The figure shows three views and two pictorial views of one solid part (mm, origin at its lowest corner). Answer the questions. Round coordinates to 2 decimals unless told otherwise and drop trailing zeros. Order: outer loops, then holes, each group sorted by start corner. A loop starts at its lowest first (then second) coordinate and runs counter-clockwise, first axis right, second up. Notation, with made-up numbers: (26.25, 83.5) - (47.25, 83.5) arc R19 cw to (47.25, 88.5) - close; hole circle Ø1 at (42, 57). An arc over 180 degrees is marked (long way). Answer as a JSON object with one key per item and string values. Group by question number.
Q1. A cutting plane is placed at C-C on y = 7.5. Determine the outline of the cut face in (x, z).
Q2. Given pin 1 Ø4 at (x, y) = (15.5, 17.5) entering from -Z, flat-ended and moving along its own axis, determine where the tip first touches the part or whether it passes through.
Q3. A cutting plane is placed at D-D on x = 20. Determine the outline of the cut face in (y, z).
Q4. A cutting plane is placed at B-B on z = 8.5. Determine the outline of the cut face in (x, y).
Q5. Consider line 1 (X direction, y = 12, z = 8.5); line 2 (X direction, y = 9.25, z = 5); line 3 (Z direction, x = 32, y = 12.25). Determine where each line is inside the solid, lowest interval first.
Q6. The mould has two halves that part along X. Classify the marked faces 1, 2, 3 and 4: pulls with the +X half, pulls with the -X half, needs draft (parallel to the pull), parting line crosses it, or undercut.
Q7. A cutting plane is placed at A-A on x = 33. Determine the outline of the cut face in (y, z), and give its area (3 significant figures).
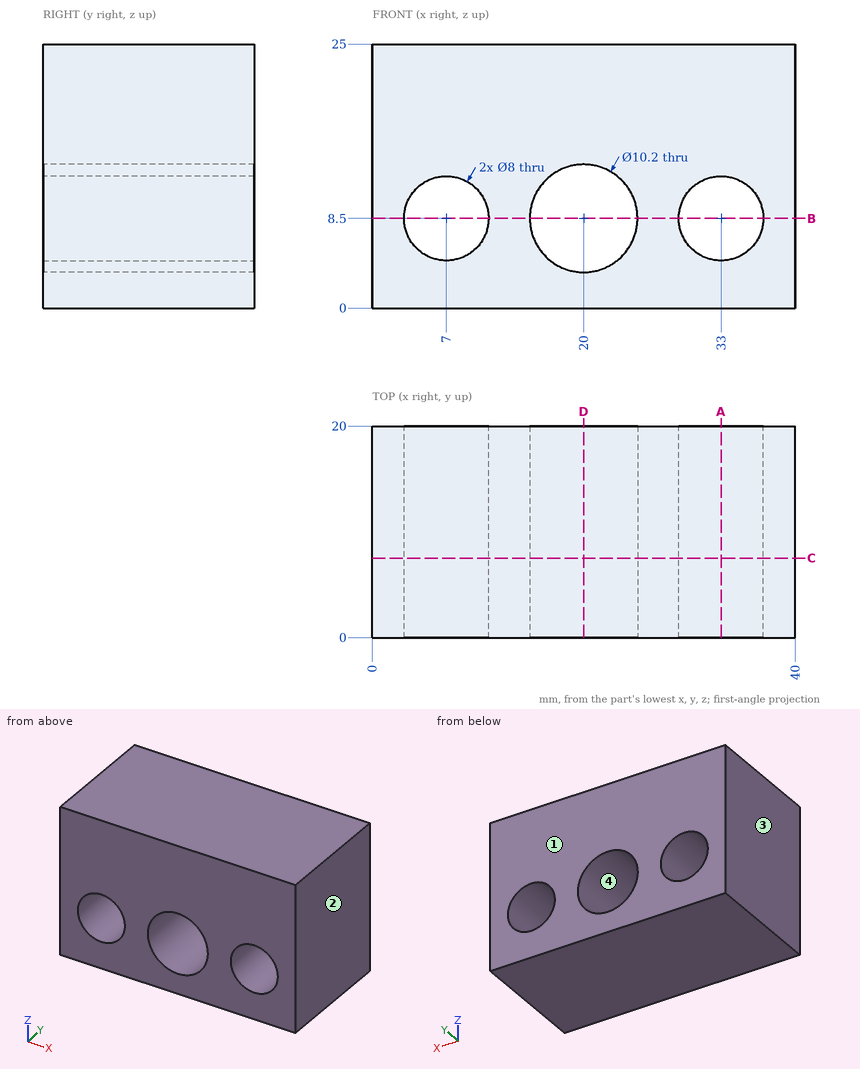
Result set:
{
 "1": {"outline": "(0, 0) - (40, 0) - (40, 25) - (0, 25) - close; hole circle Ø8 at (7, 8.5); hole circle Ø10.2 at (20, 8.5); hole circle Ø8 at (33, 8.5)"},
 "2": {"pin 1": "stops at z = 0"},
 "3": {"outline": "(0, 0) - (20, 0) - (20, 3.4) - (0, 3.4) - close; (0, 13.6) - (20, 13.6) - (20, 25) - (0, 25) - close"},
 "4": {"outline": "(0, 0) - (3, 0) - (3, 20) - (0, 20) - close; (11, 0) - (14.9, 0) - (14.9, 20) - (11, 20) - close; (25.1, 0) - (29, 0) - (29, 20) - (25.1, 20) - close; (37, 0) - (40, 0) - (40, 20) - (37, 20) - close"},
 "5": {"line 1": "x = 0 to 3, 11 to 14.9, 25.1 to 29, 37 to 40", "line 2": "x = 0 to 5.06, 8.94 to 16.29, 23.71 to 31.06, 34.94 to 40", "line 3": "z = 0 to 4.63, 12.37 to 25"},
 "6": {"face 1": "needs draft", "face 2": "pulls with the +X half", "face 3": "pulls with the -X half", "face 4": "undercut"},
 "7": {"outline": "(0, 0) - (20, 0) - (20, 4.5) - (0, 4.5) - close; (0, 12.5) - (20, 12.5) - (20, 25) - (0, 25) - close", "area": "340 mm²"}
}
